from build123d import *

# Parameters (mm, degrees)
SKETCH1_W             = 35
SKETCH1_H             = 12
BOSS_EXTRUDE1_DEPTH   = 32.2
M5_TAPPED_HOLE1_D     = 4.2
M5_TAPPED_HOLE1_DEPTH = 12.4
M5_TAPPED_HOLE1_TIP   = 1.2618073
CHAMFER2_SIZE         = 2
M4_TAPPED_HOLE1_D     = 3.3


with BuildPart() as part:
    # Sketch1 → Boss-Extrude1 (new body)
    with BuildSketch(Plane(origin=(0, 0, 0), x_dir=(1, 0, 0), z_dir=(0, 1, 0))):
        Rectangle(SKETCH1_W, SKETCH1_H)
    extrude(amount=BOSS_EXTRUDE1_DEPTH)

    # M5 Tapped Hole1
    with Locations(Plane(origin=(11.5, 32.2, 0), x_dir=(0, 0, 1), z_dir=(0, 1, 0))):
        with Locations((0, 0), (0, -18)):
            Hole(M5_TAPPED_HOLE1_D / 2, depth=M5_TAPPED_HOLE1_DEPTH)
            with Locations((0, 0, -(M5_TAPPED_HOLE1_DEPTH + M5_TAPPED_HOLE1_TIP / 2))):  # 118° drill point
                Cone(0, M5_TAPPED_HOLE1_D / 2, M5_TAPPED_HOLE1_TIP, mode=Mode.SUBTRACT)

    # Chamfer2
    chamfer2_edges = [part.edges().sort_by_distance(p)[0] for p in [
        (-17.5, 0, 0),
        (17.5, 0, 0),
    ]]
    chamfer(chamfer2_edges, length=CHAMFER2_SIZE)

    # M4 Tapped Hole1 (through all)
    with Locations(Plane(origin=(11.5, 6.9, -6), x_dir=(-1, 0, 0), z_dir=(0, 0, -1))):
        with Locations((0, 0), (22, 0)):
            Hole(M4_TAPPED_HOLE1_D / 2)


solid = part.part
Verification items for the finished model (mm, model axes). A direction names the side the tool comes from. Give positions to 0.01 mm unless a question says otherwise; leave off trailing zeros. Order: outer loops, then holes, each group sorted by start corner. A loop starts at its lowest first (then second) coordinate and runs counter-clockwise, first axis right, second up. Notation, with made-up numbers: M 48.5,30.5 L 76.5,30.5 A16 cw 76.5,50.5 Z; hole C 34,10.25 d10. An arc over 180 degrees is marked long. Answer as a JSON object with one key per item and string values. Group by question number.
1) Mould release check, pull along Z, two halves, no side actions. Record for faces 3 (the face through (0, 16, -6)), 4 (the face through (-9.739, 5.436, 0.084)), 5 (the face through (-4.418, 25.913, 0.273)): released by +Z, released by -Z, zero draft, split by the parting line, or undercut.
2) Cross-section at A-A (z = 2.75). Enter the section's corners in (x, y).
3) Access from +Z, -Z, +X, -X, +Y, -Y to the whole of each face (thin tool, end or side, straight path). Record for faces 1 (the face through (13.582, 25.913, 0.273)), 2 (the face through (16.5, 1, 0.1)).
4) Cross-section at B-B (y = 6.9). Enter the section's corners in (x, z), then the cut area to 3 significant figures.
5) Cross-section at C-C (x = -10.5). Enter the section's corners in (y, z), then the cut area to 3 significant figures.
6) Scan lines: line 1 along X through (y, z) = (28, 0); line 2 along Z through (x, y) = (-6.5, 28); line 3 along Y through (x, z) = (-10.5, -2). Record each from-to range of solid material in increasing order. Write a range as [from, to].
7) Cross-section at D-D (y = 22.5). Enter the section's corners in (x, z), then the cut area to 3 significant figures.
Result sheet:
{
 "1": {"face 3": "released by -Z", "face 4": "zero draft", "face 5": "undercut"},
 "2": {"outline": "M -17.5,2 L -15.5,0 L 15.5,0 L 17.5,2 L 17.5,32.2 L -17.5,32.2 Z; hole C -10.5,6.9 d3.3; hole C 11.5,6.9 d3.3"},
 "3": {"face 1": "+Y", "face 2": "+Z, -Z, +X, -Y"},
 "4": {"outline": "M -17.5,-6 L -12.15,-6 L -12.15,6 L -17.5,6 Z; M -8.85,-6 L 9.85,-6 L 9.85,6 L -8.85,6 Z; M 13.15,-6 L 17.5,-6 L 17.5,6 L 13.15,6 Z", "area": "341 mm2"},
 "5": {"outline": "M 0,-6 L 5.25,-6 L 5.25,6 L 0,6 Z; M 8.55,-6 L 32.2,-6 L 32.2,6 L 8.55,6 Z", "area": "347 mm2"},
 "6": {"line 1": "x = [-17.5, -8.6], [-4.4, 9.4], [13.6, 17.5]", "line 2": "z = [-6, -2.1], [2.1, 6]", "line 3": "y = [0, 5.25], [8.55, 32.2]"},
 "7": {"outline": "M -17.5,-6 L 17.5,-6 L 17.5,6 L -17.5,6 Z; hole C -6.5,0 d4.2; hole C 11.5,0 d4.2", "area": "392 mm2"}
}
